Here's how the part is built. I have some questions about the finished solid (model axes, mm). Face numbers are marked on the shaded views. Coordinates: 2 decimals unless noted, no trailing zeros. Loops run counter-clockwise (first coordinate to the right, second up) from the corner with the lowest first, then second, coordinate; pieces in that order, holes last. Notation, with made-up numbers: (46, -0.5) - (97, -0.5) arc R17 cw to (97, 9.5) - close; hole circle Ø1 at (87, 29.5). An arc over 180 degrees is marked (long way). Use a Markdown table: item, result.
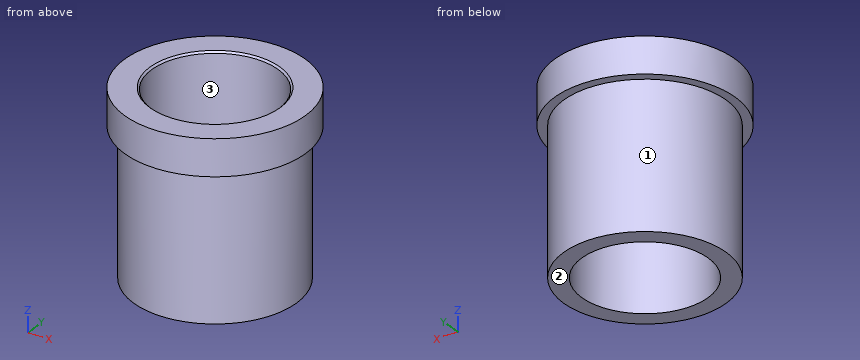
```python
from build123d import *

# Parameters (mm, degrees)
SKETCH_1_R          = 25
EXTRUDE_1_DEPTH     = 10
SKETCH_2_R          = 22.5
EXTRUDE_2_DEPTH     = 40
SKETCH_3_R          = 17.5
CUT_EXTRUDE_1_DEPTH = 80
CHAMFER_1_SIZE      = 0.5


with BuildPart() as part:
    # 草图1 → 凸台-拉伸1 (new body)
    with BuildSketch(Plane.XY):
        Circle(SKETCH_1_R)
    extrude(amount=EXTRUDE_1_DEPTH)

    # 草图2 → 凸台-拉伸2 (add)
    with BuildSketch(Plane(origin=(0, 0, 0), x_dir=(-1, 0, 0), z_dir=(0, 0, -1))):
        Circle(SKETCH_2_R)
    extrude(amount=EXTRUDE_2_DEPTH)

    # 草图3 → 切除-拉伸1 (cut)
    with BuildSketch(Plane(origin=(0, 0, -40), x_dir=(-1, 0, 0), z_dir=(0, 0, -1))):
        Circle(SKETCH_3_R)
    extrude(amount=-CUT_EXTRUDE_1_DEPTH, mode=Mode.SUBTRACT)

    # 倒角1
    chamfer_1_edges = [part.edges().sort_by_distance(p)[0] for p in [
        (17.5, 0, 10),
    ]]
    chamfer(chamfer_1_edges, length=CHAMFER_1_SIZE)


solid = part.part
```
Q1. I want a section at A-A, the plane x = 0. Write out the boundary of the cut face in (y, z), then the cut area to 3 significant figures.
Check values:
| item | result |
|---|---|
| outline | (-25, 0) - (-22.5, 0) - (-22.5, -40) - (-17.5, -40) - (-17.5, 9.5) - (-18, 10) - (-25, 10) - close; (17.5, -40) - (22.5, -40) - (22.5, 0) - (25, 0) - (25, 10) - (18, 10) - (17.5, 9.5) - close |
| area | 550 mm^2 |
Q2. Please list where these lines run through material, in increasing order: L1, parallel to Y at x = 0, z = -27.5; L2, parallel to X at y = 3.5, z = -29.5; L3, parallel to X at y = -14, z = -33. Write a range as from..to.
Check values:
| item | result |
|---|---|
| L1 | -22.5..-17.5, 17.5..22.5 |
| L2 | -22.23..-17.15, 17.15..22.23 |
| L3 | -17.61..-10.5, 10.5..17.61 |
Q3. Will these pins go through, and if not, where does the flat tip stop? P1, Ø6, axis at x = -15.5, y = 4.5, coming from the +Z side; P2, Ø2, axis at x = -12, z = -25, coming from the -Y side; P3, Ø8, axis at y = -17.5, z = -13, coming from the +X side; P4, Ø12, axis at x = 9, z = -17, coming from the -Y side.
Check values:
| item | result |
|---|---|
| P1 | z = 10 |
| P2 | y = -19.63 |
| P3 | x = 18 |
| P4 | y = -22.3 |
Q4. I want a section at C-C, the plane z = -13. Write out the boundary of the cut face in (x, y), then the cut area to 3 significant figures.
Check values:
| item | result |
|---|---|
| outline | circle Ø45 at (0, 0); hole circle Ø35 at (0, 0) |
| area | 628 mm^2 |
Q5. If we mould it in two halves opening along Y, with no side actions, what happens to the marked faces 1, 2 and 3? For each: pulls with the +Y half, pulls with the -Y half, needs draft (parallel to the pull), parting line crosses it, or undercut.
Check values:
| item | result |
|---|---|
| face 1 | parting line crosses it |
| face 2 | needs draft |
| face 3 | undercut |
